Design review of the part built by this model. Coordinates are the model's own, in mm. Face numbers are marked on the shaded views. A direction names the side the tool comes from. Round coordinates to 2 decimals unless told otherwise and drop trailing zeros. Order: outer loops, then holes, each group sorted by start corner. A loop starts at its lowest first (then second) coordinate and runs counter-clockwise, first axis right, second up. Notation, with made-up numbers: (73.25, 82) - (94.25, 82) arc R12 cw to (94.25, 102) - close; hole circle Ø1 at (-21, 45.25). An arc over 180 degrees is marked (long way). Use CSV: the item, a comma, the result in double quotes.
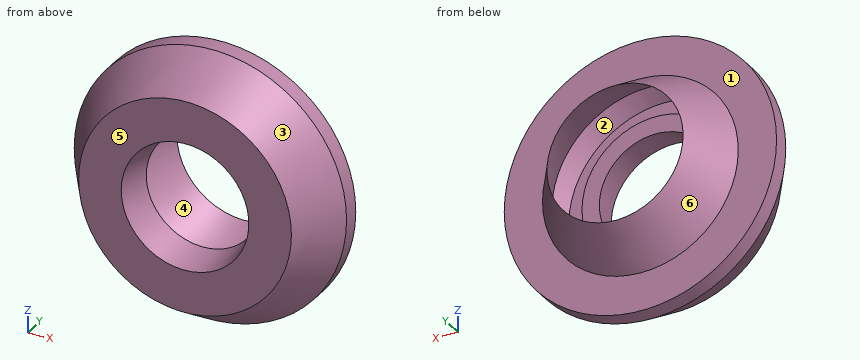
from build123d import *


with BuildPart() as part:
    # Sketch1 → Revolve1 (revolve)
    with BuildSketch(Plane.XY, mode=Mode.PRIVATE) as revolve1_sk:
        Polygon((16, 26), (23, 15), (32, 15), (32, 11), (25, 0), (15, 0), (13.45, 8), (17.524386457, 8), (18.299386457, 4), (22.804216433, 4), (27.258761887, 11), (22.994614872, 11), align=None)
    revolve(revolve1_sk.sketch.rotate(Axis((0, 12.915252942, 0), (0, -1, 0)), 180), axis=Axis((0, 12.915252942, 0), (0, -1, 0)))


solid = part.part
1) We need section C-C (y = 21.5). Give the boundary of the cut face in (x, z).
Data:
outline,"circle Ø37.73 at (0, 0); hole circle Ø36.2 at (0, 0)"
2) The part is to be moulded in two halves that separate along Z. For the marked faces 4, 5 and 6, say which applies: +Z half, -Z half, draft (parallel to the pull), parting line (faces both ways), or undercut.
Data:
face 4,"undercut"
face 5,"draft"
face 6,"parting line"
3) We need section A-A (z = 0). Give the boundary of the cut face in (x, y).
Data:
outline,"(-32, 11) - (-25, 0) - (-15, 0) - (-13.45, 8) - (-17.52, 8) - (-18.3, 4) - (-22.8, 4) - (-27.26, 11) - (-22.99, 11) - (-16, 26) - (-23, 15) - (-32, 15) - close; (13.45, 8) - (15, 0) - (25, 0) - (32, 11) - (32, 15) - (23, 15) - (16, 26) - (22.99, 11) - (27.26, 11) - (22.8, 4) - (18.3, 4) - (17.52, 8) - close"
4) For the marked faces 1, 2 and 3, list the 3-axis set-ups (+Z, -Z, +X, -X, +Y, -Y) from which the entire face can be reached by the end or side of a thin tool; tool diameter is ignored.
Data:
face 1,"+Y"
face 2,"none"
face 3,"-Y"
5) Insertion check: pin 1 Ø3 at (x, y) = (12.5, 7.5) entering from -Z; pin 2 Ø12 at (y, z) = (22.5, -1) entering from -X; pin 3 Ø12 at (x, y) = (-15, 13.5) entering from -Z. Each pin has a flat end and moves straight along its axis. Give the tip position at first contact, or say it passes through.
Data:
pin 1,"stops at z = -28.25"
pin 2,"stops at x = -22.03"
pin 3,"stops at z = -30.71"
6) We need section D-D (y = 18). Give the boundary of the cut face in (x, z), then the cut area to 3 significant figures.
Data:
outline,"circle Ø42.18 at (0, 0); hole circle Ø39.46 at (0, 0)"
area,"174 mm2"
7) We need section B-B (x = 0). Give the boundary of the cut face in (y, z), then the cut area to 3 significant figures.
Data:
outline,"(0, -25) - (11, -32) - (15, -32) - (15, -23) - (26, -16) - (11, -22.99) - (11, -27.26) - (4, -22.8) - (4, -18.3) - (8, -17.52) - (8, -13.45) - (0, -15) - close; (0, 15) - (8, 13.45) - (8, 17.52) - (4, 18.3) - (4, 22.8) - (11, 27.26) - (11, 22.99) - (26, 16) - (15, 23) - (15, 32) - (11, 32) - (0, 25) - close"
area,"292 mm2"
8) To check wall thickness, follow L1, parallel to Z at x = -3, y = 4.25; L2, parallel to Z at x = -13.5, y = 14.5; L3, parallel to Z at x = -4, y = 7.75. State the ranges of each line that lie inside material, in increasing order. Write a range as from..to.
Data:
L1,"z = -27.54..-22.77, -18..-13.86, 13.86..18, 22.77..27.54"
L2,"z = -29.01..-16.56, 16.56..29.01"
L3,"z = -29.66..-24.87, -17.11..-12.89, 12.89..17.11, 24.87..29.66"
